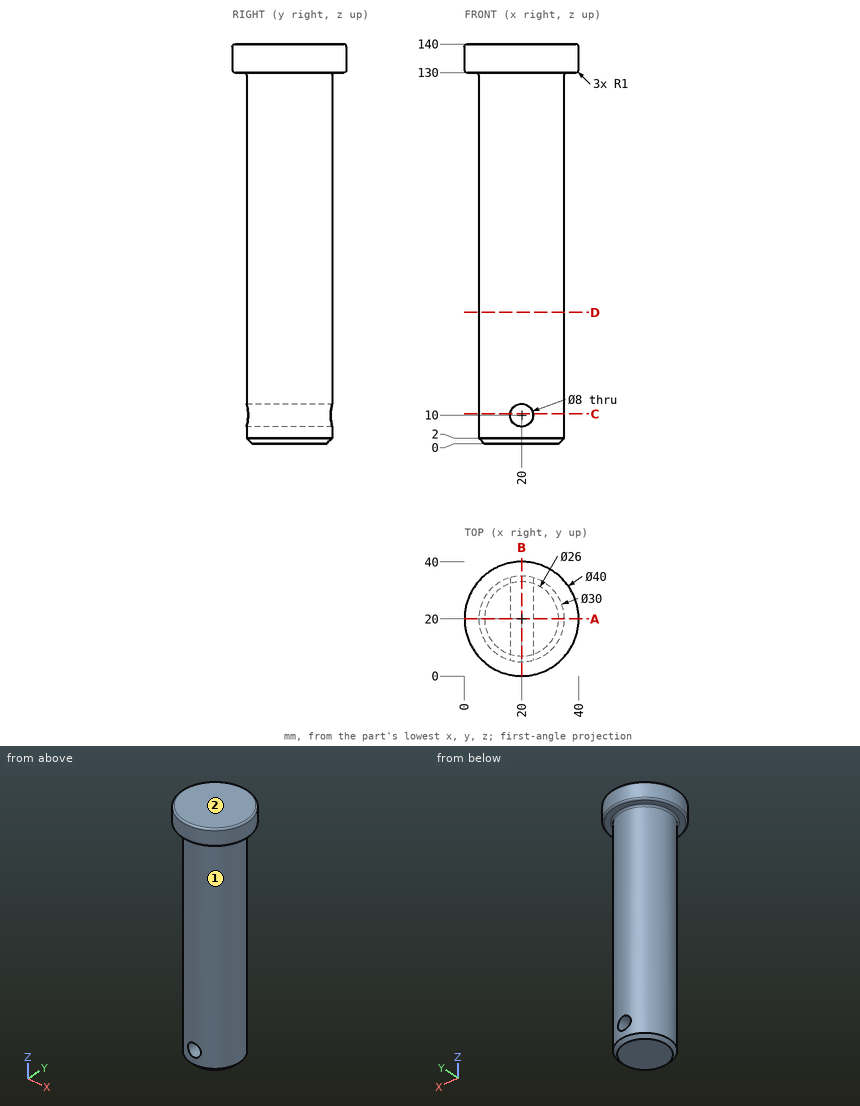
For this review, use the dimensioned drawing (mm, ordinates from the lowest corner) and the shaded views. A direction names the side the tool comes from. Round coordinates to 2 decimals unless told otherwise and drop trailing zeros. Loops run counter-clockwise (first coordinate to the right, second up) from the corner with the lowest first, then second, coordinate; pieces in that order, holes last. Notation, with made-up numbers: M -2,76 L 22,76 A21 cw 22,91 Z; hole C -32,87 d4. An arc over 180 degrees is marked long. Answer as CSV lines item,"result".
1. For the marked faces 1 and 2, list the 3-axis set-ups (+Z, -Z, +X, -X, +Y, -Y) from which the entire face can be reached by the end or side of a thin tool; tool diameter is ignored.
Outcome:
face 1,"-Z"
face 2,"+Z, +X, -X, +Y, -Y"
2. We need section A-A (y = 20). Give the boundary of the cut face in (x, z), plus the area to 3 significant figures.
Outcome:
outline,"M 0,131 A1 ccw 1,130 L 4,130 A1 cw 5,129 L 5,2 L 7,0 L 33,0 L 35,2 L 35,129 A1 cw 36,130 L 39,130 A1 ccw 40,131 L 40,139 A1 ccw 39,140 L 1,140 A1 ccw 0,139 Z; hole C 20,10 d8"
area,"4,250 mm2"
3. We need section B-B (x = 20). Give the boundary of the cut face in (y, z), plus the area to 3 significant figures.
Outcome:
outline,"M 0,131 A1 ccw 1,130 L 4,130 A1 cw 5,129 L 5,14 L 35,14 L 35,129 A1 cw 36,130 L 39,130 A1 ccw 40,131 L 40,139 A1 ccw 39,140 L 1,140 A1 ccw 0,139 Z; M 5,2 L 7,0 L 33,0 L 35,2 L 35,6 L 5,6 Z"
area,"4,060 mm2"
4. We need section C-C (z = 10.5). Give the boundary of the cut face in (x, y).
Outcome:
outline,"M 16.03,5.53 L 16.03,34.47 A15 ccw Z; M 23.97,5.53 A15 ccw 23.97,34.47 Z"
5. Insertion check: pin 1 Ø12 at (y, z) = (12.5, 108.5) entering from -X; pin 2 Ø8 at (y, z) = (26, 15) entering from +X; pin 3 Ø6 at (y, z) = (35.5, 85) entering from -X. Each pin has a flat end and moves straight along its axis. Give the tip position at first contact, or say it passes through.
Outcome:
pin 1,"stops at x = 5.08"
pin 2,"stops at x = 34.87"
pin 3,"stops at x = 11.71"
6. We need section D-D (z = 46). Give the boundary of the cut face in (x, y), plus the area to 3 significant figures.
Outcome:
outline,"C 20,20 d30"
area,"707 mm2"
7. To check wall thickness, follow L1, parallel to Z at x = 20, y = 16.5; L2, parallel to X at y = 12, z = 10; L3, parallel to Z at x = 17.5, y = 15.5. State the ranges of each line that lie inside material, in increasing order. Write a range as [from, to].
Outcome:
L1,"z = [0, 6], [14, 140]"
L2,"x = [7.31, 16], [24, 32.69]"
L3,"z = [0, 6.88], [13.12, 140]"
